```python
from build123d import *

# Parameters (mm, degrees)
SKETCH1_W                                            = 135
SKETCH1_H                                            = 80
BOSS_EXTRUDE1_DEPTH                                  = 8
CBORE_FOR_M5_HEXAGON_SOCKET_HEAD_CAP_SCR_D           = 5.5
CBORE_FOR_M5_HEXAGON_SOCKET_HEAD_CAP_SCR_CBORE_D     = 10
CBORE_FOR_M5_HEXAGON_SOCKET_HEAD_CAP_SCR_CBORE_DEPTH = 5.7
M5_TAPPED_HOLE1_D                                    = 4.2
CHAMFER1_SIZE                                        = 3
F_5_0MM_DOWEL_HOLE1_D                                = 5


with BuildPart() as part:
    # Sketch1 → Boss-Extrude1 (new body)
    with BuildSketch(Plane(origin=(0, 0, 0), x_dir=(1, 0, 0), z_dir=(0, 1, 0))):
        with Locations((67.5, 40)):
            Rectangle(SKETCH1_W, SKETCH1_H)
    extrude(amount=BOSS_EXTRUDE1_DEPTH)

    # CBORE for M5 Hexagon socket head cap screws1 (through all)
    with Locations(Plane(origin=(0, 0, 0), x_dir=(-1, 0, 0), z_dir=(0, -1, 0))):
        with Locations((-75.05, 49), (-45.05, 49), (-45.05, 7), (-75.05, 7)):
            CounterBoreHole(CBORE_FOR_M5_HEXAGON_SOCKET_HEAD_CAP_SCR_D / 2, CBORE_FOR_M5_HEXAGON_SOCKET_HEAD_CAP_SCR_CBORE_D / 2, CBORE_FOR_M5_HEXAGON_SOCKET_HEAD_CAP_SCR_CBORE_DEPTH)

    # M5 Tapped Hole1 (through all)
    with Locations(Plane(origin=(0, 8, 0), x_dir=(1, 0, 0), z_dir=(0, 1, 0))):
        with Locations((129, 25), (129, 5), (11.3, 25), (11.3, 5)):
            Hole(M5_TAPPED_HOLE1_D / 2)

    # Chamfer1
    chamfer1_edges = [part.edges().sort_by_distance(p)[0] for p in [
        (0, 4, -80),
        (135, 4, -80),
        (135, 4, 0),
        (0, 4, 0),
    ]]
    chamfer(chamfer1_edges, length=CHAMFER1_SIZE)

    # Ø5.0mm Dowel Hole1 (through all)
    with Locations(Plane(origin=(0, 0, 0), x_dir=(-1, 0, 0), z_dir=(0, -1, 0))):
        with Locations((-60.05, 7), (-60.05, 49)):
            Hole(F_5_0MM_DOWEL_HOLE1_D / 2)


solid = part.part
```
Model file for the job. Use its own axes, mm. A direction names the side the tool comes from. Give positions to 0.01 mm unless a question says otherwise; leave off trailing zeros. Loops run counter-clockwise (first coordinate to the right, second up) from the corner with the lowest first, then second, coordinate; pieces in that order, holes last. Notation, with made-up numbers: (86.25, 73.25) -> (113.25, 73.25) arc R15 cw to (113.25, 88.25) -> close; hole circle Ø7 at (-11.75, -21.5). An arc over 180 degrees is marked (long way). Use CSV: the item, a comma, the result in double quotes. Start each with the question number.
1) Wall check: line 1 (Z direction, x = 45.05, y = 6.7); line 2 (Z direction, x = 129, y = 2); line 3 (X direction, y = 2, z = -49). Give the ranges that are in metal, low to high.
2) Slice it at C-C on x = 45.05. Give the cut face in (y, z).
3) Tool access for faces 5 (the flat face through (42.9, 5.7, -4.8)), 6 (the cylindrical face through (57.552, 4.056, -7.11)): list every direction of +Z, -Z, +X, -X, +Y, -Y with a clear straight run to the whole face (end or side of a thin tool).
4) Mould opens along Z. For faces 1 (the flat face through (67, 4, 0)), 2 (the flat face through (2, 4, -79)), 3 (the cylindrical face through (9.297, 3.944, -5.631)), 4 (the flat face through (67, 8, -41)) say: released by +Z, released by -Z, zero draft, split by the parting line, or undercut.
5) Slice it at D-D on x = 60.05. Give the cut face in (y, z), plus the area to 3 significant figures.
6) Slice it at A-A on x = 129. Give the cut face in (y, z).
7) Slice it at B-B on y = 2. Give the number of separate pieces and of enclosed holes in the cut face, plus the area to 3 significant figures.
8) Flat gauge pins, fed straight in: pin 1 Ø11 at (x, z) = (75.5, -47) entering from -Y; pin 2 Ø9 at (x, z) = (45.05, -49) entering from -Y. Where does each tip first touch, or does it go through?
Computed values:
1,line 1,"z = -80 to -51.75, -46.25 to -9.75, -4.25 to 0"
1,line 2,"z = -80 to -27.1, -22.9 to -7.1, -2.9 to 0"
1,line 3,"x = 0 to 40.05, 50.05 to 57.55, 62.55 to 70.05, 80.05 to 135"
2,outline,"(0, -80) -> (8, -80) -> (8, -51.75) -> (5.7, -51.75) -> (5.7, -54) -> (0, -54) -> close; (0, -44) -> (5.7, -44) -> (5.7, -46.25) -> (8, -46.25) -> (8, -9.75) -> (5.7, -9.75) -> (5.7, -12) -> (0, -12) -> close; (0, -2) -> (5.7, -2) -> (5.7, -4.25) -> (8, -4.25) -> (8, 0) -> (0, 0) -> close"
3,face 5,"-Y"
3,face 6,"+Y, -Y"
4,face 1,"released by +Z"
4,face 2,"released by -Z"
4,face 3,"undercut"
4,face 4,"zero draft"
5,outline,"(0, -80) -> (8, -80) -> (8, -51.5) -> (0, -51.5) -> close; (0, -46.5) -> (8, -46.5) -> (8, -9.5) -> (0, -9.5) -> close; (0, -4.5) -> (8, -4.5) -> (8, 0) -> (0, 0) -> close"
5,area,"560 mm^2"
6,outline,"(0, -80) -> (8, -80) -> (8, -27.1) -> (0, -27.1) -> close; (0, -22.9) -> (8, -22.9) -> (8, -7.1) -> (0, -7.1) -> close; (0, -2.9) -> (8, -2.9) -> (8, 0) -> (0, 0) -> close"
7,separate pieces,"1"
7,enclosed holes,"10"
7,area,"10,400 mm^2"
8,pin 1,"stops at y = 0"
8,pin 2,"stops at y = 5.7"
